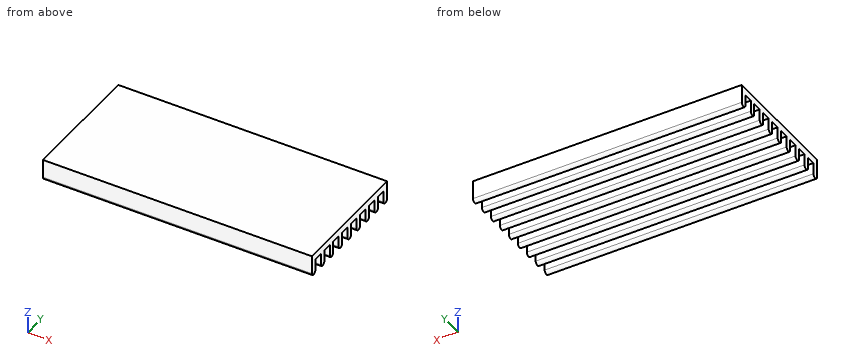
```python
from build123d import *

# Parameters (mm, degrees)
SKETCH_1_W             = 75
SKETCH_1_H             = 35
EXTRUDE_1_DEPTH        = 6
SKETCH_2_W             = 75
SKETCH_2_H             = 2.55
CUT_EXTRUDE_1_DEPTH    = 4
PATTERN_LINEAR_1_COUNT = 8
PATTERN_LINEAR_1_PITCH = 4.17
FILLET_2_RADIUS        = 0.81
FILLET_2_LENGTH        = 75
FILLET_3_RADIUS        = 0.81
FILLET_3_LENGTH        = 75
FILLET_4_RADIUS        = 0.81
FILLET_4_LENGTH        = 75
FILLET_5_RADIUS        = 0.81
FILLET_5_LENGTH        = 75
FILLET_6_RADIUS        = 0.81
FILLET_6_LENGTH        = 75
FILLET_7_RADIUS        = 0.81
FILLET_7_LENGTH        = 75
FILLET_8_RADIUS        = 0.81
FILLET_8_LENGTH        = 75
FILLET_9_RADIUS        = 0.81
FILLET_9_LENGTH        = 75
FILLET_10_RADIUS       = 0.82
FILLET_10_LENGTH       = 75


with BuildPart() as part:
    # 草图1 → 拉伸1 (new body)
    with BuildSketch(Plane.XY):
        Rectangle(SKETCH_1_W, SKETCH_1_H)
    extrude(amount=EXTRUDE_1_DEPTH)

    # 草图2 → 切除-拉伸1 (cut)
    with BuildSketch(Plane(origin=(0, 0, 0), x_dir=(-1, 0, 0), z_dir=(0, 0, -1))):
        with Locations((0, 14.605)):
            Rectangle(SKETCH_2_W, SKETCH_2_H)
    cut_extrude_1 = extrude(amount=-CUT_EXTRUDE_1_DEPTH, mode=Mode.SUBTRACT)

    # 阵列(线性)1: 切除-拉伸1 ×8
    with Locations(*[(0, -i * PATTERN_LINEAR_1_PITCH, 0) for i in range(1, PATTERN_LINEAR_1_COUNT)]):
        add(cut_extrude_1, mode=Mode.SUBTRACT)

    # 圆角2: full round fillet: the end face becomes a half cylinder, R = half its width
    fillet_2_face = Plane((0, 16.69, 0), x_dir=(-1, 0, 0), z_dir=(0, 0, -1))  # on the end face: x along it, z out of the body
    fillet_2_slab = fillet_2_face.offset(-FILLET_2_RADIUS / 2) * Box(FILLET_2_LENGTH, 2 * FILLET_2_RADIUS, FILLET_2_RADIUS, mode=Mode.PRIVATE)  # the body's end, R deep
    fillet_2_round = Plane((0, 16.69, 0.81), x_dir=(0, 0, -1), z_dir=(-1, 0, 0)) * Cylinder(FILLET_2_RADIUS, FILLET_2_LENGTH, mode=Mode.PRIVATE)  # its axis R under the face
    add(fillet_2_slab - fillet_2_round, mode=Mode.SUBTRACT)

    # 圆角3: full round fillet: the end face becomes a half cylinder, R = half its width
    fillet_3_face = Plane((0, 12.52, 0), x_dir=(1, 0, 0), z_dir=(0, 0, -1))  # on the end face: x along it, z out of the body
    fillet_3_slab = fillet_3_face.offset(-FILLET_3_RADIUS / 2) * Box(FILLET_3_LENGTH, 2 * FILLET_3_RADIUS, FILLET_3_RADIUS, mode=Mode.PRIVATE)  # the body's end, R deep
    fillet_3_round = Plane((0, 12.52, 0.81), x_dir=(0, 0, -1), z_dir=(1, 0, 0)) * Cylinder(FILLET_3_RADIUS, FILLET_3_LENGTH, mode=Mode.PRIVATE)  # its axis R under the face
    add(fillet_3_slab - fillet_3_round, mode=Mode.SUBTRACT)

    # 圆角4: full round fillet: the end face becomes a half cylinder, R = half its width
    fillet_4_face = Plane((0, 8.35, 0), x_dir=(1, 0, 0), z_dir=(0, 0, -1))  # on the end face: x along it, z out of the body
    fillet_4_slab = fillet_4_face.offset(-FILLET_4_RADIUS / 2) * Box(FILLET_4_LENGTH, 2 * FILLET_4_RADIUS, FILLET_4_RADIUS, mode=Mode.PRIVATE)  # the body's end, R deep
    fillet_4_round = Plane((0, 8.35, 0.81), x_dir=(0, 0, -1), z_dir=(1, 0, 0)) * Cylinder(FILLET_4_RADIUS, FILLET_4_LENGTH, mode=Mode.PRIVATE)  # its axis R under the face
    add(fillet_4_slab - fillet_4_round, mode=Mode.SUBTRACT)

    # 圆角5: full round fillet: the end face becomes a half cylinder, R = half its width
    fillet_5_face = Plane((0, 4.18, 0), x_dir=(1, 0, 0), z_dir=(0, 0, -1))  # on the end face: x along it, z out of the body
    fillet_5_slab = fillet_5_face.offset(-FILLET_5_RADIUS / 2) * Box(FILLET_5_LENGTH, 2 * FILLET_5_RADIUS, FILLET_5_RADIUS, mode=Mode.PRIVATE)  # the body's end, R deep
    fillet_5_round = Plane((0, 4.18, 0.81), x_dir=(0, 0, -1), z_dir=(1, 0, 0)) * Cylinder(FILLET_5_RADIUS, FILLET_5_LENGTH, mode=Mode.PRIVATE)  # its axis R under the face
    add(fillet_5_slab - fillet_5_round, mode=Mode.SUBTRACT)

    # 圆角6: full round fillet: the end face becomes a half cylinder, R = half its width
    fillet_6_face = Plane((0, 0.01, 0), x_dir=(1, 0, 0), z_dir=(0, 0, -1))  # on the end face: x along it, z out of the body
    fillet_6_slab = fillet_6_face.offset(-FILLET_6_RADIUS / 2) * Box(FILLET_6_LENGTH, 2 * FILLET_6_RADIUS, FILLET_6_RADIUS, mode=Mode.PRIVATE)  # the body's end, R deep
    fillet_6_round = Plane((0, 0.01, 0.81), x_dir=(0, 0, -1), z_dir=(1, 0, 0)) * Cylinder(FILLET_6_RADIUS, FILLET_6_LENGTH, mode=Mode.PRIVATE)  # its axis R under the face
    add(fillet_6_slab - fillet_6_round, mode=Mode.SUBTRACT)

    # 圆角7: full round fillet: the end face becomes a half cylinder, R = half its width
    fillet_7_face = Plane((0, -4.16, 0), x_dir=(1, 0, 0), z_dir=(0, 0, -1))  # on the end face: x along it, z out of the body
    fillet_7_slab = fillet_7_face.offset(-FILLET_7_RADIUS / 2) * Box(FILLET_7_LENGTH, 2 * FILLET_7_RADIUS, FILLET_7_RADIUS, mode=Mode.PRIVATE)  # the body's end, R deep
    fillet_7_round = Plane((0, -4.16, 0.81), x_dir=(0, 0, -1), z_dir=(1, 0, 0)) * Cylinder(FILLET_7_RADIUS, FILLET_7_LENGTH, mode=Mode.PRIVATE)  # its axis R under the face
    add(fillet_7_slab - fillet_7_round, mode=Mode.SUBTRACT)

    # 圆角8: full round fillet: the end face becomes a half cylinder, R = half its width
    fillet_8_face = Plane((0, -8.33, 0), x_dir=(-1, 0, 0), z_dir=(0, 0, -1))  # on the end face: x along it, z out of the body
    fillet_8_slab = fillet_8_face.offset(-FILLET_8_RADIUS / 2) * Box(FILLET_8_LENGTH, 2 * FILLET_8_RADIUS, FILLET_8_RADIUS, mode=Mode.PRIVATE)  # the body's end, R deep
    fillet_8_round = Plane((0, -8.33, 0.81), x_dir=(0, 0, -1), z_dir=(-1, 0, 0)) * Cylinder(FILLET_8_RADIUS, FILLET_8_LENGTH, mode=Mode.PRIVATE)  # its axis R under the face
    add(fillet_8_slab - fillet_8_round, mode=Mode.SUBTRACT)

    # 圆角9: full round fillet: the end face becomes a half cylinder, R = half its width
    fillet_9_face = Plane((0, -12.5, 0), x_dir=(1, 0, 0), z_dir=(0, 0, -1))  # on the end face: x along it, z out of the body
    fillet_9_slab = fillet_9_face.offset(-FILLET_9_RADIUS / 2) * Box(FILLET_9_LENGTH, 2 * FILLET_9_RADIUS, FILLET_9_RADIUS, mode=Mode.PRIVATE)  # the body's end, R deep
    fillet_9_round = Plane((0, -12.5, 0.81), x_dir=(0, 0, -1), z_dir=(1, 0, 0)) * Cylinder(FILLET_9_RADIUS, FILLET_9_LENGTH, mode=Mode.PRIVATE)  # its axis R under the face
    add(fillet_9_slab - fillet_9_round, mode=Mode.SUBTRACT)

    # 圆角10: full round fillet: the end face becomes a half cylinder, R = half its width
    fillet_10_face = Plane((0, -16.68, 0), x_dir=(1, 0, 0), z_dir=(0, 0, -1))  # on the end face: x along it, z out of the body
    fillet_10_slab = fillet_10_face.offset(-FILLET_10_RADIUS / 2) * Box(FILLET_10_LENGTH, 2 * FILLET_10_RADIUS, FILLET_10_RADIUS, mode=Mode.PRIVATE)  # the body's end, R deep
    fillet_10_round = Plane((0, -16.68, 0.82), x_dir=(0, 0, -1), z_dir=(1, 0, 0)) * Cylinder(FILLET_10_RADIUS, FILLET_10_LENGTH, mode=Mode.PRIVATE)  # its axis R under the face
    add(fillet_10_slab - fillet_10_round, mode=Mode.SUBTRACT)


solid = part.part
```
Could you check a few things on this model? Use its own coordinates, in mm. Round coordinates to 2 decimals unless told otherwise and drop trailing zeros. Loops run counter-clockwise (first coordinate to the right, second up) from the corner with the lowest first, then second, coordinate; pieces in that order, holes last. Notation, with made-up numbers: M 80,72 L 93,72 A21 ccw 93,92 Z; hole C -19,68.5 d5. An arc over 180 degrees is marked long. Write item = value, one per line.
1. I need wall thicknesses on probe 1 along Z at (x, y) = (23.5, -10); probe 2 along Z at (x, y) = (-31, -13). Which ranges of each line are inside material? Lowest first, please.
Results below:
probe_1 = 4 to 6
probe_2 = 0.17 to 6
2. I want a section at B-B, the plane y = 11. Write out the boundary of the cut face in (x, z), and give its area (3 significant figures).
Results below:
outline = M -37.5,4 L 37.5,4 L 37.5,6 L -37.5,6 Z
area = 150 mm²
3. I want a section at A-A, the plane z = 2.1. Count the separate pieces of the cut face and the enclosed holes in it, and give its area (4 significant figures).
Results below:
separate_pieces = 9
enclosed_holes = 0
area = 1,095 mm²
4. Will these pins go through, and if not, where does the flat tip stop? P1, Ø2, axis at x = -27, y = 4, coming from the -Z side; P2, Ø2, axis at x = -15, y = 10.5, coming from the -Z side.
Results below:
P1 = 0
P2 = 4
